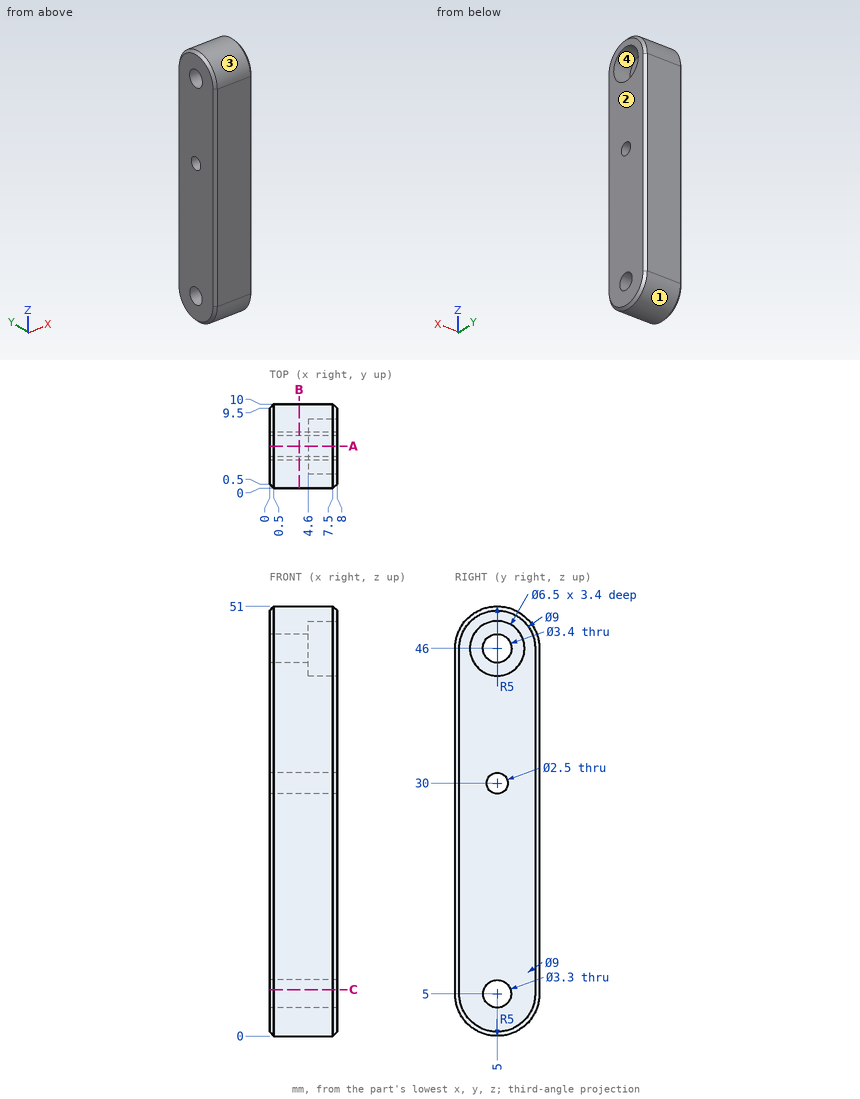
Study the drawing (mm; zero at the part's minimum x, y, z) and answer. Round coordinates to 2 decimals unless told otherwise and drop trailing zeros. Write each loop counter-clockwise with the first axis right and the second up, starting at its lowest first coordinate (ties: lowest second). Pieces come first, ordered by that corner, then holes. Notation, with made-up numbers: (-27, -29.75) -> (16, -29.75) arc R18 ccw to (16, -23.75) -> close; hole circle Ø1 at (80.5, 74). An arc over 180 degrees is marked (long way). Write each question's results on one line, items separated by ' | '.
Item 1: A cutting plane is placed at B-B, the plane x = 3.5. Determine the outline of the cut face in (y, z).
Result set:
outline: (0, 5) arc R5 ccw to (10, 5) -> (10, 46) arc R5 ccw to (0, 46) -> close; hole circle Ø3.4 at (5, 46); hole circle Ø3.3 at (5, 5); hole circle Ø2.5 at (5, 30)
Item 2: Find the intervals of material crossed by line 1 along Y through (x, z) = (1.4, 46); line 2 along Y through (x, z) = (3.5, 30); line 3 along Z through (x, y) = (4.75, 6.5), in increasing order. Write a range as [from, to].
Result set:
line 1: [0, 3.3], [6.7, 10] | line 2: [0, 3.75], [6.25, 10] | line 3: [0.23, 4.31], [5.69, 43.12], [48.88, 50.77]
Item 3: A cutting plane is placed at A-A, the plane y = 5. Determine the outline of the cut face in (x, z).
Result set:
outline: (0, 0.5) -> (0.5, 0) -> (7.5, 0) -> (8, 0.5) -> (8, 3.35) -> (0, 3.35) -> close; (0, 6.65) -> (8, 6.65) -> (8, 28.75) -> (0, 28.75) -> close; (0, 31.25) -> (8, 31.25) -> (8, 42.75) -> (4.6, 42.75) -> (4.6, 44.3) -> (0, 44.3) -> close; (0, 47.7) -> (4.6, 47.7) -> (4.6, 49.25) -> (8, 49.25) -> (8, 50.5) -> (7.5, 51) -> (0.5, 51) -> (0, 50.5) -> close
Item 4: Flat-ended cylindrical pins translate along their axes: P1, Ø2.5, axis at y = 5, z = 5, coming from the +X side; P2, Ø3, axis at y = 6.5, z = 45.5, coming from the +X side; P3, Ø3, axis at x = 4, y = 1.5, coming from the -Z side. Find the tip coordinate at first contact, or state that the pin passes through.
Result set:
P1: through | P2: x = 4.6 | P3: z = 0.42
Item 5: The mould has two halves that part along Z. Classify the marked faces 1, 2, 3 and 4: +Z half, -Z half, draft (parallel to the pull), parting line (faces both ways), or undercut.
Result set:
face 1: -Z half | face 2: draft | face 3: +Z half | face 4: undercut
Item 6: A cutting plane is placed at C-C, the plane z = 5.5. Determine the outline of the cut face in (x, y), plus the area to 3 significant figures.
Result set:
outline: (0, 0.5) -> (0.5, 0) -> (7.5, 0) -> (8, 0.5) -> (8, 3.43) -> (0, 3.43) -> close; (0, 6.57) -> (8, 6.57) -> (8, 9.5) -> (7.5, 10) -> (0.5, 10) -> (0, 9.5) -> close | area: 54.3 mm^2
